```python
from build123d import *

# Parameters (mm, degrees)
SKETCH_2_R          = 17.5
CUT_EXTRUDE_1_DEPTH = 10
SKETCH_3_R          = 7.5
CUT_EXTRUDE_2_DEPTH = 10


with BuildPart() as part:
    # 草图1 → 旋转1 (revolve)
    with BuildSketch(Plane(origin=(0, 0, 0), x_dir=(0, 0, -1), z_dir=(1, 0, 0))):
        Polygon((0, 0), (0, 130), (9, 130), (11.75, 21), (32.5, 17), (32.5, 0), align=None)
    revolve(axis=Axis((0, 0, 0), (0, 1, 0)))

    # 草图2 → 切除-拉伸1 (cut)
    with BuildSketch(Plane.XZ):
        with Locations(Location((0, 0, 0), (0, 0, 270))):
            Circle(SKETCH_2_R)
    extrude(amount=-CUT_EXTRUDE_1_DEPTH, mode=Mode.SUBTRACT)

    # 草图3 → 切除-拉伸2 (cut)
    with BuildSketch(Plane.XZ.offset(-10)):
        with Locations(Location((0, 0, 0), (0, 0, 270))):
            Circle(SKETCH_3_R)
    extrude(amount=-CUT_EXTRUDE_2_DEPTH, mode=Mode.SUBTRACT)


solid = part.part
```
Geometry: final body of the model. Coordinates: model frame, mm. A direction names the side the tool comes from. Round coordinates to 2 decimals unless told otherwise and drop trailing zeros. Loops run counter-clockwise (first coordinate to the right, second up) from the corner with the lowest first, then second, coordinate; pieces in that order, holes last. Notation, with made-up numbers: (84.5, 20) -> (136.5, 20) arc R14 ccw to (136.5, 42) -> close; hole circle Ø7 at (27, 21). An arc over 180 degrees is marked (long way). Use one line per item in the form item = value. Start each with the question number.
1) Line query: L1, parallel to X at y = 7, z = 0; L2, parallel to X at y = 15.5, z = 0; L3, parallel to Y at x = 7, z = -23. Output: solid intervals per line, ascending.
2) Section A-A on x = 0. Output: boundary loops of the cut face in (y, z).
3) Draft query along X for faces 1 (the flat face through (14, 0, -14)), 2 (the conical face through (12.74, 20.75, 2.83)), 3 (the flat face through (-8, 10, 0)). Return one class per face: released by +X, released by -X, zero draft, split by the parting line, or undercut.
4) Section D-D on y = 53. Output: boundary loops of the cut face in (x, z), then the cut area to 3 significant figures.
5) Section C-C on y = 72. Output: boundary loops of the cut face in (x, z), then the cut area to 3 significant figures.
6) Section B-B on z = 0. Output: boundary loops of the cut face in (x, y), then the cut area to 3 significant figures.
7) Access query for faces 4 (the conical face through (6.32, 74.74, 8.25)), 5 (the cylindrical face through (-9.76, 8.38, -31)), 6 (the cylindrical face through (0.33, 14.93, 7.493)). Directions: +Z, -Z, +X, -X, +Y, -Y. A direction counts if a zero-diameter tool reaches every point of the face in a straight line with its end or side. Return the directions, or none.
8) First-contact query: P1, Ø10, axis at x = -24, z = -24, coming from the -Y side; P2, Ø7.5, axis at x = 3, z = -1, coming from the -Y side; P3, Ø1.5, axis at x = 7.5, y = 34.5, coming from the -Z side; P4, Ø8, axis at y = 26.5, z = 21.5, coming from the -X side. Flat tips, straight axial feed; report the tip coordinate or a pass-through.
Response:
q1.L1 = -32.5 to -17.5, 17.5 to 32.5
q1.L2 = -32.5 to -7.5, 7.5 to 32.5
q1.L3 = 0 to 18.63
q2.outline = (0, -32.5) -> (17, -32.5) -> (21, -11.75) -> (130, -9) -> (130, 9) -> (21, 11.75) -> (17, 32.5) -> (0, 32.5) -> (0, 17.5) -> (10, 17.5) -> (10, 7.5) -> (20, 7.5) -> (20, -7.5) -> (10, -7.5) -> (10, -17.5) -> (0, -17.5) -> close
q3.face_1 = zero draft
q3.face_2 = split by the parting line
q3.face_3 = undercut
q4.outline = circle Ø21.89 at (0, 0)
q4.area = 376 mm^2
q5.outline = circle Ø20.93 at (0, 0)
q5.area = 344 mm^2
q6.outline = (-32.5, 0) -> (-17.5, 0) -> (-17.5, 10) -> (-7.5, 10) -> (-7.5, 20) -> (7.5, 20) -> (7.5, 10) -> (17.5, 10) -> (17.5, 0) -> (32.5, 0) -> (32.5, 17) -> (11.75, 21) -> (9, 130) -> (-9, 130) -> (-11.75, 21) -> (-32.5, 17) -> close
q6.area = 3,040 mm^2
q7.face_4 = +Y
q7.face_5 = +Y, -Y
q7.face_6 = -Y
q8.P1 = 0
q8.P2 = 20
q8.P3 = -9.2
q8.P4 = through
